The figure shows three views and two pictorial views of one solid part (mm, origin at its lowest corner). Answer the questions. A direction names the side the tool comes from. Coordinates: 2 decimals unless noted, no trailing zeros. Order: outer loops, then holes, each group sorted by start corner. A loop starts at its lowest first (then second) coordinate and runs counter-clockwise, first axis right, second up.
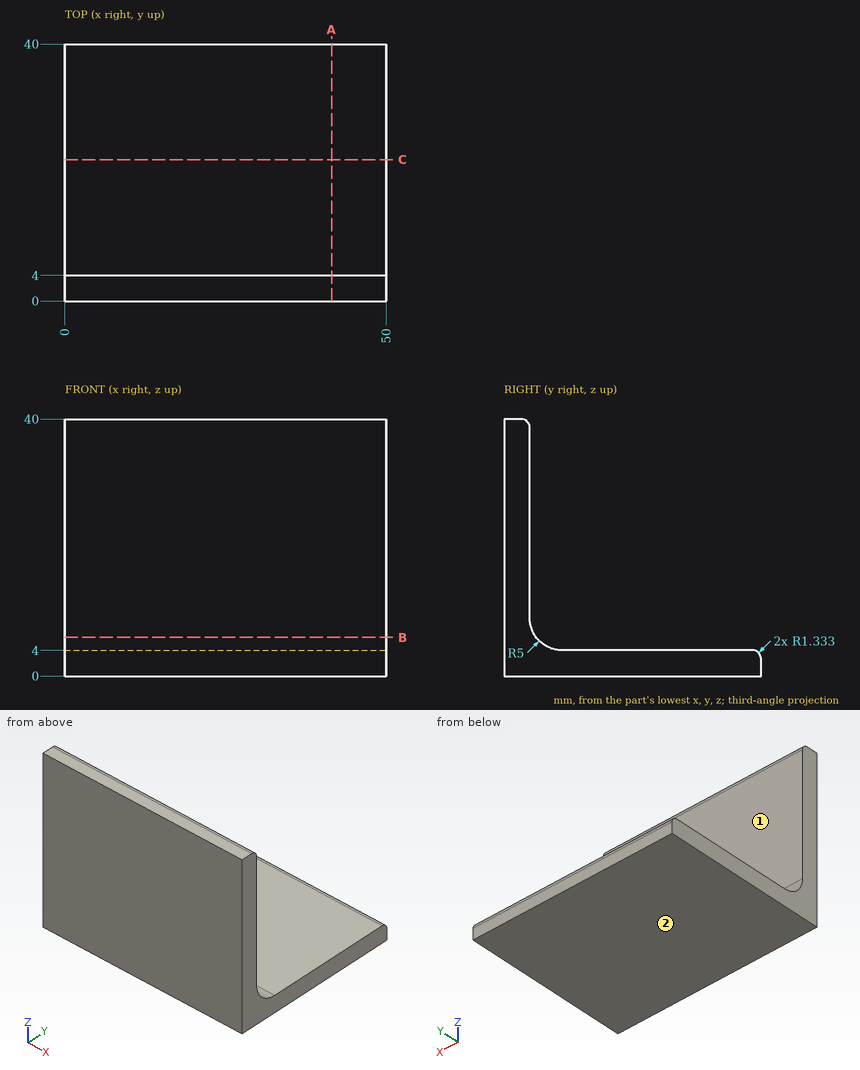
1) Each of these flat-tipped pins is pushed along its axis until it touches: P1, Ø2, axis at x = 22.5, y = 35.5, coming from the -Z side; P2, Ø23.5, axis at x = 32, y = 25.5, coming from the +Z side; P3, Ø1, axis at x = 34, z = 8.5, coming from the +Y side; P4, Ø9, axis at x = 32, z = 27.5, coming from the +Y side. Where does it stop, or does it pass through?
2) A cutting plane is placed at B-B, the plane z = 6. Write down the section's boundary in (x, y).
3) For the marked faces 1 and 2, determine the directions among +Z, -Z, +X, -X, +Y, -Y from which every point of the face is accessible in a straight line to the end or side of a thin tool.
4) A cutting plane is placed at A-A, the plane x = 41.5. Write down the section's boundary in (y, z).
5) Straight lines are drawn through the part: probe 1 along Y at (x, z) = (26, 28); probe 2 along Y at (x, z) = (18.5, 7.5). For each, find the intervals that lie inside material, in ascending order.
6) A cutting plane is placed at C-C, the plane y = 22. Write down the section's boundary in (x, z).
Working result:
1. P1: stops at z = 0
1. P2: stops at z = 4
1. P3: stops at y = 4.1
1. P4: stops at y = 4
2. outline: (0, 0) - (50, 0) - (50, 5) - (0, 5) - close
3. face 1: +Z, +X, -X, +Y
3. face 2: -Z, +X, -X, +Y, -Y
4. outline: (0, 0) - (40, 0) - (40, 2.67) arc R1.33 ccw to (38.67, 4) - (9, 4) arc R5 cw to (4, 9) - (4, 38.67) arc R1.33 ccw to (2.67, 40) - (0, 40) - close
5. probe 1: y = 0 to 4
5. probe 2: y = 0 to 4.23
6. outline: (0, 0) - (50, 0) - (50, 4) - (0, 4) - close
